```python
from build123d import *

# Parameters (mm, degrees)
SKETCH_1_W                  = 25
SKETCH_1_H                  = 900
EXTRUDE_1_DEPTH             = 25
CUT_EXTRUDE_1_DEPTH         = 901.694176733
CHAMFER_1_SIZE              = 0.5
HOLE_WIZARD_1_D             = 5.5
HOLE_WIZARD_1_CBORE_D       = 9
HOLE_WIZARD_1_CBORE_DEPTH   = 15
HOLE_WIZARD_M5_1_AT_2_COUNT = 2
HOLE_WIZARD_M5_1_AT_2_PITCH = 60
PATTERN_LINEAR_1_COUNT      = 2
PATTERN_LINEAR_1_PITCH      = 285


with BuildPart() as part:
    # 草图1 → 拉伸1 (new body)
    with BuildSketch(Plane(origin=(0, 0, 0), x_dir=(0, 0, -1), z_dir=(1, 0, 0))):
        with Locations((12.5, 450)):
            Rectangle(SKETCH_1_W, SKETCH_1_H)
    extrude(amount=EXTRUDE_1_DEPTH)

    # 草图2 → 切除-拉伸1 (cut, through all)
    with BuildSketch(Plane.XZ):
        with BuildLine():
            Line((0, -7.5), (6.5, -7.5))
            ThreePointArc((6.5, -7.5), (7.207106781, -7.792893219), (7.5, -8.5))
            Line((7.5, -8.5), (7.5, -16.5))
            ThreePointArc((7.5, -16.5), (7.207106781, -17.207106781), (6.5, -17.5))
            Line((6.5, -17.5), (0, -17.5))
            Line((0, -17.5), (0, -7.5))
        make_face()
    extrude(amount=-CUT_EXTRUDE_1_DEPTH, mode=Mode.SUBTRACT)

    # 倒角1
    chamfer_1_edges = [part.edges().sort_by_distance(p)[0] for p in [
        (0, 450, -17.5),
        (0, 450, -7.5),
    ]]
    chamfer(chamfer_1_edges, length=CHAMFER_1_SIZE)

    # 孔1 (through all)
    with Locations(Plane(origin=(12.5, 887.5, 0), x_dir=(1, 0, 0), z_dir=(0, 0, 1))):
        with Locations((0, 0), (0, -875)):
            CounterBoreHole(HOLE_WIZARD_1_D / 2, HOLE_WIZARD_1_CBORE_D / 2, HOLE_WIZARD_1_CBORE_DEPTH)

    # 草图5 → M5 螺纹孔1 (revolve, cut)
    with BuildSketch(Plane(origin=(12.5, 622, 0), x_dir=(0, -1, 0), z_dir=(1, 0, 0))):
        Polygon((0, 0), (0, 13.6618073), (2.1, 12.4), (2.1, 10), (2.5, 10), (2.5, 0), align=None)
    hole_wizard_m5_1 = revolve(axis=Axis((12.5, 622, 6.35), (0, 0, -1)), mode=Mode.SUBTRACT)

    # M5 螺纹孔1 at 2: M5 螺纹孔1 ×2
    with Locations(*[(0, -i * HOLE_WIZARD_M5_1_AT_2_PITCH, 0) for i in range(1, HOLE_WIZARD_M5_1_AT_2_COUNT)]):
        add(hole_wizard_m5_1, mode=Mode.SUBTRACT)

    # 阵列(线性)1: M5 螺纹孔1 ×2
    with Locations(*[(0, -i * PATTERN_LINEAR_1_PITCH, 0) for i in range(1, PATTERN_LINEAR_1_COUNT)]):
        add(hole_wizard_m5_1, mode=Mode.SUBTRACT)

    # 阵列(线性)1 copy 1 sketch → 阵列(线性)1 copy 1 (revolve, cut)
    with BuildSketch(Plane(origin=(12.5, 277, 0), x_dir=(0, -1, 0), z_dir=(1, 0, 0))):
        Polygon((0, 0), (0, 13.6618073), (2.1, 12.4), (2.1, 10), (2.5, 10), (2.5, 0), align=None)
    revolve(axis=Axis((12.5, 277, 6.35), (0, 0, -1)), mode=Mode.SUBTRACT)


solid = part.part
```
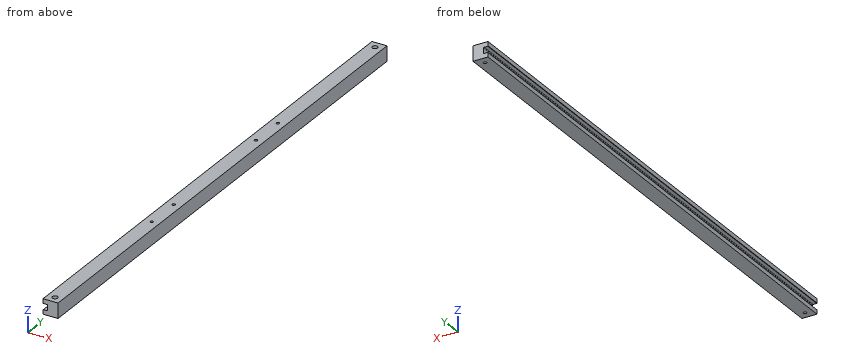
CAD build for the part. Positions are in the model's coordinates, mm. Give positions to 0.01 mm unless a question says otherwise; leave off trailing zeros. Write each loop counter-clockwise with the first axis right and the second up, starting at its lowest first coordinate (ties: lowest second). Pieces come first, ordered by that corner, then holes. Notation, with made-up numbers: M -31,46 L -5,46 A12 cw -5,62 Z; hole C 46,-21 d6. An arc over 180 degrees is marked long. Return JSON: item names as keys, results as strings. Group by question number.
(1) Band-saw the part on A-A (y = 96). Give the cut face in (x, z), and give its area (3 significant figures).
(2) Drill centre lines: L1, parallel to Y at x = 12.5, z = -19; L2, parallel to Z at x = 2, y = 166; L3, parallel to X at y = 887.5, z = -18.5. Where is each one in solid material? Low to high. Write a range as [from, to].
(3) Flat gauge pins, fed straight in: pin 1 Ø2.5 at (x, y) = (12.5, 337) entering from +Z; pin 2 Ø1.5 at (x, y) = (11.5, 337.5) entering from +Z; pin 3 Ø1.5 at (x, y) = (13, 621.5) entering from +Z. Where does each tip first touch, or does it go through?
Entries:
{
 "1": {"outline": "M 0,-25 L 25,-25 L 25,0 L 0,0 L 0,-7 L 0.5,-7.5 L 6.5,-7.5 A1 cw 7.5,-8.5 L 7.5,-16.5 A1 cw 6.5,-17.5 L 0.5,-17.5 L 0,-18 Z", "area": "550 mm^2"},
 "2": {"L1": "y = [0, 9.75], [15.25, 884.75], [890.25, 900]", "L2": "z = [-25, -17.5], [-7.5, 0]", "L3": "x = [0, 9.75], [15.25, 25]"},
 "3": {"pin 1": "stops at z = -12.91", "pin 2": "stops at z = -12.54", "pin 3": "stops at z = -12.79"}
}
